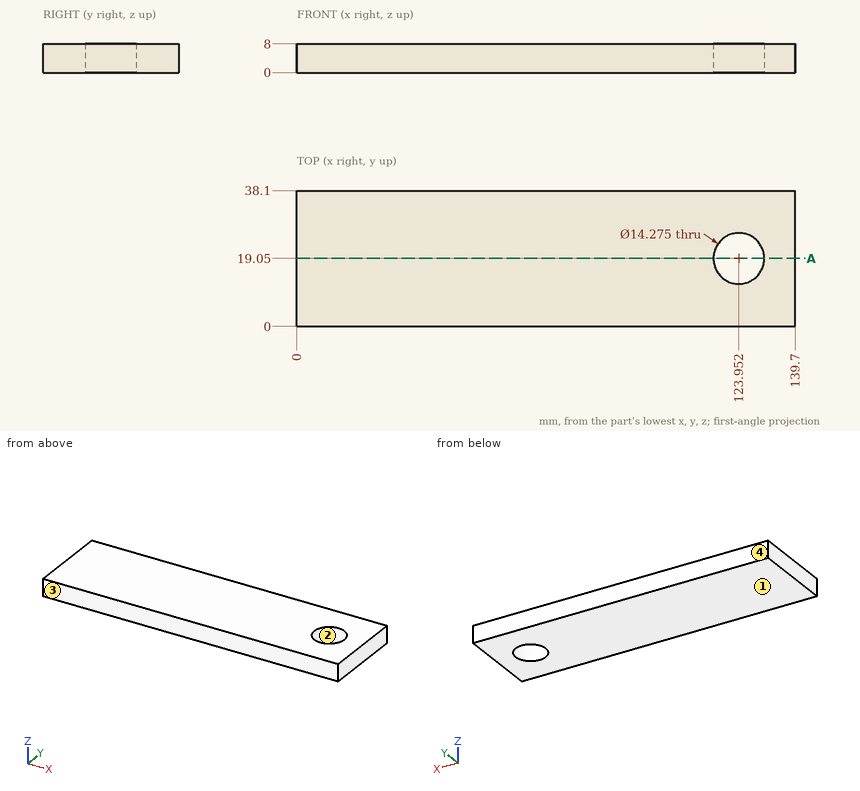
Input: dimensioned drawing with shaded views. Units: mm. Origin: part minimum x, y, z. Give positions to 0.01 mm unless a question says otherwise; leave off trailing zeros. Order: outer loops, then holes, each group sorted by start corner. A loop starts at its lowest first (then second) coordinate and runs counter-clockwise, first axis right, second up.
(1) Material intervals for line 1 along Y through (x, z) = (130.5, 1); line 2 along Y through (x, z) = (125, 6.5); line 3 along X through (y, z) = (20, 2), sorted ascending.
(2) Pull-direction query (Y, two-part tool) for the marked faces 1, 2, 3 and 4; classes: +Y half, -Y half, draft (parallel to the pull), parting line (faces both ways), or undercut.
(3) Section query A-A (y = 19.05). Return the cut outline in (x, z) (1 decimal), plus the area to 3 significant figures.
(4) Contact query for a flat-ended pin moving along its axis: P1, Ø13, axis at x = 123.952, y = 19.05, coming from the +Z side. Output: stop coordinate, or through.
Outcome:
1. line 1: y = 0 to 16.21, 21.89 to 38.1
1. line 2: y = 0 to 11.99, 26.11 to 38.1
1. line 3: x = 0 to 116.88, 131.03 to 139.7
2. face 1: draft
2. face 2: undercut
2. face 3: -Y half
2. face 4: +Y half
3. outline: (0, 0) - (116.8, 0) - (116.8, 8) - (0, 8) - close; (131.1, 0) - (139.7, 0) - (139.7, 8) - (131.1, 8) - close
3. area: 1,000 mm2
4. P1: passes through
